from build123d import *

# Parameters (mm, degrees)
BASE_PLATE_DEPTH   = 1
WEB_SKETCH_W       = 3
WEB_SKETCH_H       = 1
WEB_DEPTH          = 4
LUG_DEPTH          = 1
LUG_HOLES_SKETCH_R = 0.75
LUG_HOLES_2X_DEPTH = 1
WEB_FILLET_R0_5_R  = 0.5


with BuildPart() as part:
    # Base Plate Sketch → Base Plate (new body)
    with BuildSketch(Plane.XY):
        with BuildLine():
            Line((-3, 4.5), (3, 4.5))
            Line((3, 4.5), (3, 3.5))
            ThreePointArc((3, 3.5), (2, 2.5), (3, 1.5))
            Line((3, 1.5), (3, -1.5))
            ThreePointArc((3, -1.5), (2, -2.5), (3, -3.5))
            Line((3, -3.5), (3, -4.5))
            Line((3, -4.5), (-3, -4.5))
            Line((-3, -4.5), (-3, -3.5))
            ThreePointArc((-3, -3.5), (-2, -2.5), (-3, -1.5))
            Line((-3, -1.5), (-3, 1.5))
            ThreePointArc((-3, 1.5), (-2, 2.5), (-3, 3.5))
            Line((-3, 3.5), (-3, 4.5))
        make_face()
    extrude(amount=BASE_PLATE_DEPTH)

    # Web Sketch → Web (add)
    with BuildSketch(Plane.XY.offset(1)):
        Rectangle(WEB_SKETCH_W, WEB_SKETCH_H)
    extrude(amount=WEB_DEPTH)

    # Lug Sketch → Lug (add)
    with BuildSketch(Plane.XY.offset(5)):
        with BuildLine():
            Line((1.5, 3), (1.5, -3))
            ThreePointArc((1.5, -3), (0, -4.5), (-1.5, -3))
            Line((-1.5, -3), (-1.5, 3))
            ThreePointArc((-1.5, 3), (0, 4.5), (1.5, 3))
        make_face()
    extrude(amount=LUG_DEPTH)

    # Lug Holes Sketch → Lug Holes 2x (cut)
    with BuildSketch(Plane.XY.offset(6)):
        with Locations((0, 3)):
            Circle(LUG_HOLES_SKETCH_R)
        with Locations((0, -3)):
            Circle(LUG_HOLES_SKETCH_R)
    extrude(amount=-LUG_HOLES_2X_DEPTH, mode=Mode.SUBTRACT)

    # Web Fillet R0.5
    web_fillet_r0_5_edges = [part.edges().sort_by_distance(p)[0] for p in [
        (1.5, 0, 1),
        (-1.5, 0, 1),
    ]]
    fillet(web_fillet_r0_5_edges, radius=WEB_FILLET_R0_5_R)


solid = part.part
Model file for the job. Use its own axes, mm. A direction names the side the tool comes from. Give positions to 0.01 mm unless a question says otherwise; leave off trailing zeros. Write each loop counter-clockwise with the first axis right and the second up, starting at its lowest first coordinate (ties: lowest second). Pieces come first, ordered by that corner, then holes. Notation, with made-up numbers: M -25,52.25 L -11,52.25 A10 cw -11,68.25 Z; hole C 43,64 d4. An arc over 180 degrees is marked long. One line per item, written item: value. Start each with the question number.
Q1. 3-axis set-ups, long thin cutter, end or side, ignore diameter. For faces 1 (the cylindrical face through (0, 4.5, 5.5)), 2 (the flat face through (-3, 4, 0.5)): which of +Z, -Z, +X, -X, +Y, -Y reach the whole face in a straight line?
Q2. Saw through at A-A, the plane x = 0. Write the cut outline in (y, z).
Q3. Saw through at C-C, the plane y = -2.5. Write the cut outline in (x, z).
Q4. Saw through at D-D, the plane x = 0.9. Write the cut outline in (y, z).
Q5. Saw through at B-B, the plane z = 5.35. Write the cut outline in (x, y).
Q6. Drop flat-ended pins along their axis: pin 1 Ø3.5 at (y, z) = (0.5, 4) entering from -X; pin 2 Ø1 at (y, z) = (-2.5, 4) entering from -X; pin 3 Ø3 at (x, z) = (-0.5, 3) entering from +Y. Give the stop position or say it passes through.
Q7. Probe probe 1 along Y at (x, z) = (0, 5.4); probe 2 along Z at (x, y) = (0.8, 3.75); probe 3 along Y at (x, z) = (0.65, 3.9). List the from-to ranges inside material, lowest first. Write a range as [from, to].
Q8. Two-plate mould, pull along Z, no slides. Class faces 3 (the flat face through (0, 0, 0)), 4 (the cylindrical face through (-0.163, -3.732, 5.507)), 5 (the flat face through (0, 0.5, 3)), 6 (the flat face through (0, -2, 5)): +Z half, -Z half, draft (parallel to the pull), parting line (faces both ways), or undercut.
Output values:
1. face 1: +Z, +Y
1. face 2: +Z, -Z, -X, +Y, -Y
2. outline: M -4.5,0 L 4.5,0 L 4.5,1 L 0.5,1 L 0.5,5 L 2.25,5 L 2.25,6 L -2.25,6 L -2.25,5 L -0.5,5 L -0.5,1 L -4.5,1 Z; M -4.5,5 L -3.75,5 L -3.75,6 L -4.5,6 Z; M 3.75,5 L 4.5,5 L 4.5,6 L 3.75,6 Z
3. outline: M -2,0 L 2,0 L 2,1 L -2,1 Z; M -1.5,5 L -0.56,5 L -0.56,6 L -1.5,6 Z; M 0.56,5 L 1.5,5 L 1.5,6 L 0.56,6 Z
4. outline: M -4.5,0 L 4.5,0 L 4.5,1 L 0.5,1 L 0.5,5 L 4.2,5 L 4.2,6 L -4.2,6 L -4.2,5 L -0.5,5 L -0.5,1 L -4.5,1 Z
5. outline: M -1.5,-3 A1.5 ccw 1.5,-3 L 1.5,3 A1.5 ccw -1.5,3 Z; hole C 0,-3 d1.5; hole C 0,3 d1.5
6. pin 1: stops at x = -1.5
6. pin 2: passes through
6. pin 3: stops at y = 0.5
7. probe 1: y = [-4.5, -3.75], [-2.25, 2.25], [3.75, 4.5]
7. probe 2: z = [0, 1], [5, 6]
7. probe 3: y = [-0.5, 0.5]
8. face 3: -Z half
8. face 4: draft
8. face 5: undercut
8. face 6: undercut
